Read the model definition and answer for the solid it produces. Units are mm, in the model's axes. A direction names the side the tool comes from. Coordinates: 2 decimals unless noted, no trailing zeros. Write each loop counter-clockwise with the first axis right and the second up, starting at its lowest first coordinate (ties: lowest second). Pieces come first, ordered by that corner, then holes.
(1) The mould has two halves that part along X. Classify faces 3 (the flat face through (0, -17.5, 0)), 4 (the flat face through (25, -1, 0)), 5 (the cylindrical face through (-22.493, 10.105, -0.33)), 6 (the flat face through (20, 2.5, 0)): +X half, -X half, draft (parallel to the pull), parting line (faces both ways), or undercut.
(2) Section C-C on y = 4 is taken. Write down the section's boundary in (x, z).
(3) Find the intervals of material crossed by probe 1 along Z at (x, y) = (15, 13); probe 2 along X at (y, z) = (-0.5, 1.5); probe 3 along Z at (x, y) = (15, -5), in increasing order.
(4) Section A-A on z = 0 is taken. Write down the section's boundary in (x, y).
(5) Given pin 1 (12 mm diameter, centred on x = 15, z = 0, fed in from +Y); pin 2 (4 mm diameter, centred on x = 12.5, z = 7, fed in from +Y), each flat-ended and moving along its own axis, determine where each tip first touches the part or whether it passes through.
(6) Section D-D on z = 6 is taken. Write down the section's boundary in (x, y).
(7) Section B-B on x = 15 is taken. Write down the section's boundary in (y, z).
(8) Which of the six approach directions +Z, -Z, +X, -X, +Y, -Y give full straight-line access (tool end or side, diameter ignored) to faces 1 (the cylindrical face through (19.496, -7.64, -0.198)), 2 (the flat face through (-15, 2.5, 5))?
from build123d import *

# Parameters (mm, degrees)
SKETCH_2_W                   = 50
SKETCH_2_H                   = 35
EXTRUDE_1_DEPTH              = 10
HOLE_WIZARD_M8_1_D           = 9
HOLE_WIZARD_M8_1_CBORE_D     = 15
HOLE_WIZARD_M8_1_CBORE_DEPTH = 15
CHAMFER_1_SIZE               = 2


with BuildPart() as part:
    # 草图2 → 凸台-拉伸1 (new, symmetric)
    with BuildSketch(Plane.XY):
        Rectangle(SKETCH_2_W, SKETCH_2_H)
    extrude(amount=EXTRUDE_1_DEPTH, both=True)

    # M8 六角凹头螺钉的柱形沉头孔1 (through all)
    with Locations(Plane(origin=(0, 17.5, 0), x_dir=(1, 0, 0), z_dir=(0, 1, 0))):
        with Locations((15, 0), (-15, 0)):
            CounterBoreHole(HOLE_WIZARD_M8_1_D / 2, HOLE_WIZARD_M8_1_CBORE_D / 2, HOLE_WIZARD_M8_1_CBORE_DEPTH)

    # 倒角1
    chamfer_1_edges = [part.edges().sort_by_distance(p)[0] for p in [
        (-25, 17.5, 0),
        (25, 17.5, 0),
    ]]
    chamfer(chamfer_1_edges, length=CHAMFER_1_SIZE)


solid = part.part
Response:
1. face 3: draft
1. face 4: +X half
1. face 5: undercut
1. face 6: undercut
2. outline: (-25, -10) - (25, -10) - (25, 10) - (-25, 10) - close; hole circle Ø15 at (-15, 0); hole circle Ø15 at (15, 0)
3. probe 1: z = -10 to -7.5, 7.5 to 10
3. probe 2: x = -25 to -19.24, -10.76 to 10.76, 19.24 to 25
3. probe 3: z = -10 to -4.5, 4.5 to 10
4. outline: (-25, -17.5) - (-19.5, -17.5) - (-19.5, 2.5) - (-22.5, 2.5) - (-22.5, 17.5) - (-23, 17.5) - (-25, 15.5) - close; (-10.5, -17.5) - (10.5, -17.5) - (10.5, 2.5) - (7.5, 2.5) - (7.5, 17.5) - (-7.5, 17.5) - (-7.5, 2.5) - (-10.5, 2.5) - close; (19.5, -17.5) - (25, -17.5) - (25, 15.5) - (23, 17.5) - (22.5, 17.5) - (22.5, 2.5) - (19.5, 2.5) - close
5. pin 1: stops at y = 2.5
5. pin 2: stops at y = 17.5
6. outline: (-25, -17.5) - (25, -17.5) - (25, 15.5) - (23, 17.5) - (19.5, 17.5) - (19.5, 2.5) - (10.5, 2.5) - (10.5, 17.5) - (-10.5, 17.5) - (-10.5, 2.5) - (-19.5, 2.5) - (-19.5, 17.5) - (-23, 17.5) - (-25, 15.5) - close
7. outline: (-17.5, -10) - (17.5, -10) - (17.5, -7.5) - (2.5, -7.5) - (2.5, -4.5) - (-17.5, -4.5) - close; (-17.5, 4.5) - (2.5, 4.5) - (2.5, 7.5) - (17.5, 7.5) - (17.5, 10) - (-17.5, 10) - close
8. face 1: +Y, -Y
8. face 2: +Y
